Geometry: final body of the model. Coordinates: model frame, mm. Give positions to 0.01 mm unless a question says otherwise; leave off trailing zeros. Loops run counter-clockwise (first coordinate to the right, second up) from the corner with the lowest first, then second, coordinate; pieces in that order, holes last.
from build123d import *

# Parameters (mm, degrees)
LUG_PROFILE_SKETCH_R = 25
LUG_PLATE_20MM_DEPTH = 20


with BuildPart() as part:
    # Lug Profile Sketch → Lug Plate 20mm (new body)
    with BuildSketch(Plane.XY):
        with BuildLine():
            Line((-140, -240), (140, -240))
            Line((140, -240), (47.017565913, 17.010246783))
            ThreePointArc((47.017565913, 17.010246783), (0, 50), (-47.017565913, 17.010246783))
            Line((-47.017565913, 17.010246783), (-140, -240))
        make_face()
        Circle(LUG_PROFILE_SKETCH_R, mode=Mode.SUBTRACT)
    extrude(amount=LUG_PLATE_20MM_DEPTH)


solid = part.part
Item 1: Section query A-A on x = 0. Return loops of the section in (y, z), plus the area to 3 significant figures.
Values follow:
outline: (-240, 0) - (-25, 0) - (-25, 20) - (-240, 20) - close; (25, 0) - (50, 0) - (50, 20) - (25, 20) - close
area: 4,800 mm2
Item 2: Ray query, probe 1 along X at (y, z) = (-8, 3); probe 2 along X at (y, z) = (-16.5, 6); probe 3 along X at (y, z) = (-218.5, 17). Return the intervals inside material, ascending.
Values follow:
probe 1: x = -56.07 to -23.69, 23.69 to 56.07
probe 2: x = -59.14 to -18.78, 18.78 to 59.14
probe 3: x = -132.22 to 132.22
Item 3: Draft query along Y for faces 1 (the face through (23.846, 7.509, 9.86)), 2 (the face through (-2, -125, 0)), 3 (the face through (-2, -240, 10)). Return one class per face: +Y half, -Y half, draft (parallel to the pull), parting line (faces both ways), or undercut.
Values follow:
face 1: undercut
face 2: draft
face 3: -Y half
Item 4: Section query D-D on x = -78. Return loops of the section in (y, z), plus the area to 3 significant figures.
Values follow:
outline: (-240, 0) - (-68.63, 0) - (-68.63, 20) - (-240, 20) - close
area: 3,430 mm2
Item 5: Section query B-B on z = 3.75. Return loops of the section in (x, y).
Values follow:
outline: (-140, -240) - (140, -240) - (47.02, 17.01) arc R50 ccw to (-47.02, 17.01) - close; hole circle Ø50 at (0, 0)
Item 6: Pin query (flat end, axial travel): pin 1 (1.5 mm diameter, centred on y = -116.5, z = 12, fed in from -X); pin 2 (12 mm diameter, centred on y = -124, z = 15.5, fed in from +X); pin 3 (3 mm diameter, centred on y = -194.5, z = 2.5, fed in from -X). Return the tip coordinate at first contact, or that it passes through.
Values follow:
pin 1: stops at x = -95.59
pin 2: stops at x = 100.2
pin 3: stops at x = -124.08
Item 7: Section query C-C on y = 0. Return loops of the section in (x, z), plus the area to 3 significant figures.
Values follow:
outline: (-53.17, 0) - (-25, 0) - (-25, 20) - (-53.17, 20) - close; (25, 0) - (53.17, 0) - (53.17, 20) - (25, 20) - close
area: 1,130 mm2
